Part print with two shaded views. Sizes in mm from the minimum x, y, z corner. A direction names the side the tool comes from. Coordinates: 2 decimals unless noted, no trailing zeros. Write each loop counter-clockwise with the first axis right and the second up, starting at its lowest first coordinate (ties: lowest second). Pieces come first, ordered by that corner, then holes. Notation, with made-up numbers: (2.5, 31.25) - (26.5, 31.25) arc R21 cw to (26.5, 65.25) - close; hole circle Ø7 at (26, 67). An arc over 180 degrees is marked (long way). Answer in a Markdown table with one row per item. Add a question column.
Q1. Band-saw the part on A-A (z = 7.25). List the corners of the cut face in (x, y), and give its area (3 significant figures).
Q2. Band-saw the part on B-B (y = 23). List the corners of the cut face in (x, z), and give its area (3 significant figures).
Q3. Band-saw the part on C-C (z = 14.75). List the corners of the cut face in (x, y), and give its area (3 significant figures).
Q4. Pin check, flat tips, straight feed: pin 1 (8 mm diameter, centred on x = 27.5, y = 7.5, fed in from +Z); pin 2 (5 mm diameter, centred on x = 4.5, z = 4.5, fed in from -Y); pin 3 (8 mm diameter, centred on x = 15.5, z = 2.5, fed in from +Y); pin 4 (17.5 mm diameter, centred on x = 20, y = 25, fed in from -Z). Stop position of each tip, or through.
Q5. 3-axis set-ups, long thin cutter, end or side, ignore diameter. For the marked faces 4, 5 and 6: which of +Z, -Z, +X, -X, +Y, -Y reach the whole face in a straight line?
Q6. Band-saw the part on D-D (x = 7.5). List the corners of the cut face in (y, z).
Q7. Drill centre lines: line 1 along Y through (x, z) = (27.5, 10.5); line 2 along Z through (x, y) = (33.5, 17.5); line 3 along Y through (x, z) = (27.5, 5.75). Where is each one in solid material? Low to high. Write a range as from..to.
Q8. Two-plate mould, pull along Y, no slides. Class the marked faces 1, 2 and 3: +Y half, -Y half, draft (parallel to the pull), parting line (faces both ways), or undercut.
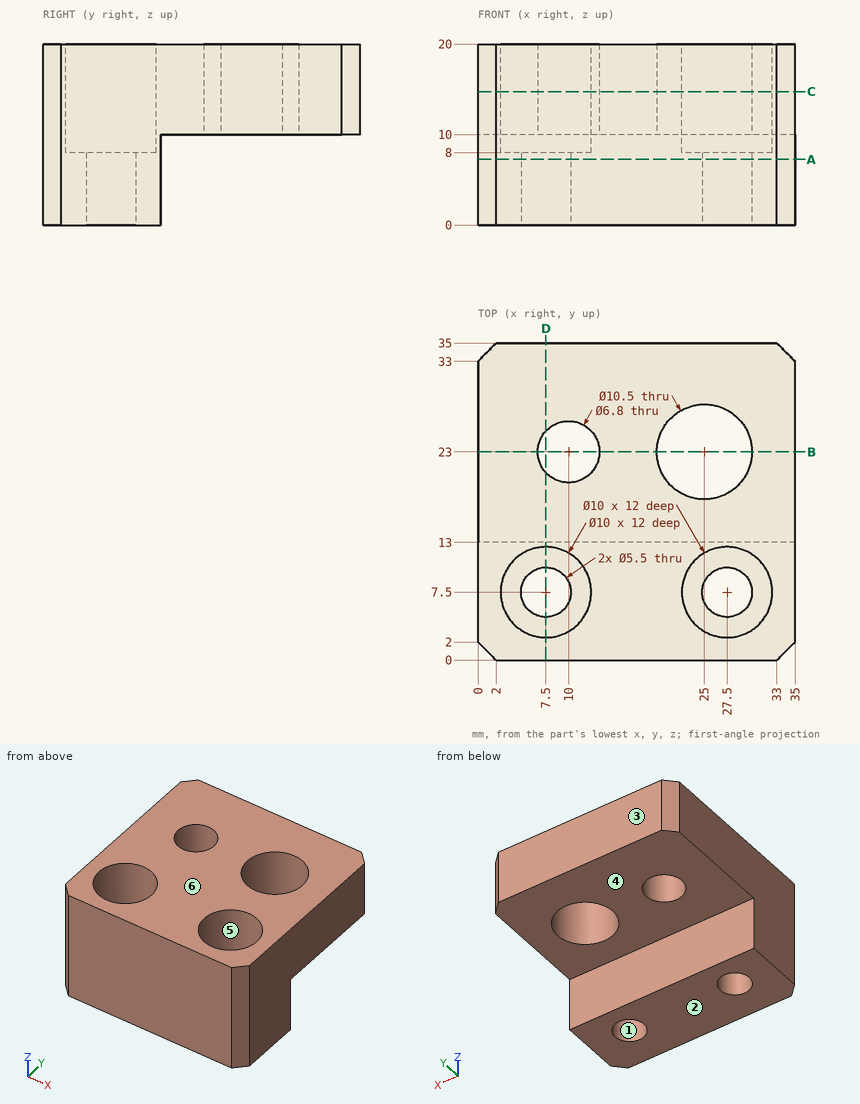
Checked values:
| question | item | result |
|---|---|---|
| 1 | outline | (0, 2) - (2, 0) - (33, 0) - (35, 2) - (35, 13) - (0, 13) - close; hole circle Ø5.5 at (7.5, 7.5); hole circle Ø5.5 at (27.5, 7.5) |
| 1 | area | 403 mm² |
| 2 | outline | (0, 10) - (6.6, 10) - (6.6, 20) - (0, 20) - close; (13.4, 10) - (19.75, 10) - (19.75, 20) - (13.4, 20) - close; (30.25, 10) - (35, 10) - (35, 20) - (30.25, 20) - close |
| 2 | area | 177 mm² |
| 3 | outline | (0, 2) - (2, 0) - (33, 0) - (35, 2) - (35, 33) - (33, 35) - (2, 35) - (0, 33) - close; hole circle Ø10 at (7.5, 7.5); hole circle Ø6.8 at (10, 23); hole circle Ø10.5 at (25, 23); hole circle Ø10 at (27.5, 7.5) |
| 3 | area | 937 mm² |
| 4 | pin 1 | stops at z = 8 |
| 4 | pin 2 | stops at y = 0 |
| 4 | pin 3 | stops at y = 13 |
| 4 | pin 4 | stops at z = 10 |
| 5 | face 4 | -Z, +X, -X, +Y |
| 5 | face 5 | +Z |
| 5 | face 6 | +Z, +X, -X, +Y, -Y |
| 6 | outline | (0, 0) - (4.75, 0) - (4.75, 8) - (2.5, 8) - (2.5, 20) - (0, 20) - close; (10.25, 0) - (13, 0) - (13, 10) - (20.7, 10) - (20.7, 20) - (12.5, 20) - (12.5, 8) - (10.25, 8) - close; (25.3, 10) - (35, 10) - (35, 20) - (25.3, 20) - close |
| 7 | line 1 | y = 0..2.5, 12.5..18.38, 27.62..35 |
| 7 | line 2 | z = 10..20 |
| 7 | line 3 | y = 0..4.75, 10.25..13 |
| 8 | face 1 | undercut |
| 8 | face 2 | draft |
| 8 | face 3 | +Y half |
